```python
from build123d import *

# Parameters (mm, degrees)
FORKED_BLOCK_BODY_DEPTH      = 42.5
SLOT_12X24_DEPTH             = 85
RELIEF_GROOVE_SKETCH_W       = 72
RELIEF_GROOVE_SKETCH_H       = 6
BOTTOM_RELIEF_GROOVE_6_DEPTH = 50
BORE_AND_SADDLE_SKETCH_R     = 12
SADDLE_RECESS_48_DEPTH       = 12
BORE_24_REACH                = 177.873
SKETCH6_3_R                  = 12


with BuildPart() as part:
    # Block Profile Sketch → Forked Block Body (new, symmetric)
    with BuildSketch(Plane(origin=(0, 0, 0), x_dir=(0, 0, -1), z_dir=(1, 0, 0))):
        Polygon((50, 0), (-95, 0), (-95, 90), (-59, 90), (-59, 25), (50, 25), align=None)
    extrude(amount=FORKED_BLOCK_BODY_DEPTH, both=True)

    # Slot Sketch → Slot 12x24 (cut)
    with BuildSketch(Plane(origin=(0, 25, 0), x_dir=(1, 0, 0), z_dir=(0, 1, 0))):
        with BuildLine():
            Line((18.5, 0), (18.5, 50))
            Line((18.5, 50), (-5.5, 50))
            Line((-5.5, 50), (-5.5, 0))
            ThreePointArc((-5.5, 0), (6.5, -12), (18.5, 0))
        make_face()
    extrude(amount=-SLOT_12X24_DEPTH, mode=Mode.SUBTRACT)

    # Relief Groove Sketch → Bottom Relief Groove 6 (cut)
    with BuildSketch(Plane(origin=(42.5, 0, 0), x_dir=(0, 0, -1), z_dir=(1, 0, 0))):
        with Locations((-59, 3)):
            Rectangle(RELIEF_GROOVE_SKETCH_W, RELIEF_GROOVE_SKETCH_H)
    extrude(amount=-BOTTOM_RELIEF_GROOVE_6_DEPTH, mode=Mode.SUBTRACT)

    # Bore and Saddle Sketch → Saddle Recess _48 (cut)
    with BuildSketch(Plane.XY.offset(95)):
        with BuildLine():
            Line((-42.5, 66), (-42.5, 30))
            Line((-42.5, 30), (-24, 30))
            ThreePointArc((-24, 30), (0, 18), (24, 30))
            Line((24, 30), (42.5, 30))
            Line((42.5, 30), (42.5, 66))
            Line((42.5, 66), (24, 66))
            ThreePointArc((24, 66), (0, 78), (-24, 66))
            Line((-24, 66), (-42.5, 66))
        make_face()
        with Locations((0, 48)):
            Circle(BORE_AND_SADDLE_SKETCH_R, mode=Mode.SUBTRACT)
    extrude(amount=-SADDLE_RECESS_48_DEPTH, mode=Mode.SUBTRACT)

    # Sketch6_3 → Bore _24 (cut, up to next)
    with BuildSketch(Plane.XY.offset(95), mode=Mode.PRIVATE) as bore_24_sk1:
        with Locations((0, 48)):
            Circle(SKETCH6_3_R)
    bore_24_tool1 = extrude(bore_24_sk1.sketch, amount=-BORE_24_REACH, mode=Mode.PRIVATE) & part.part
    add(bore_24_tool1.solids().sort_by_distance((0, 48, 95))[0], mode=Mode.SUBTRACT)


solid = part.part
```
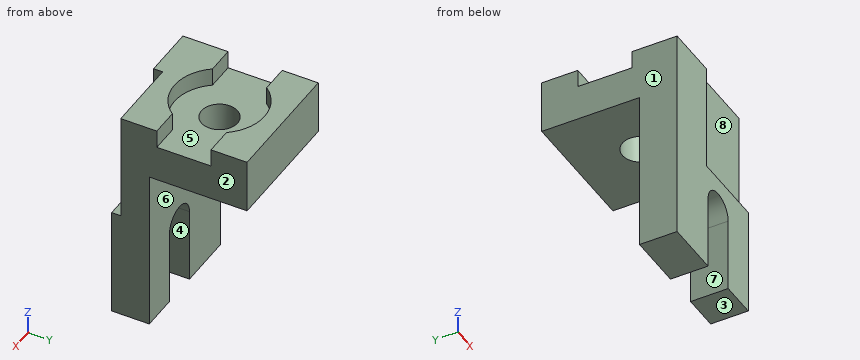
Design review of the part built by this model. Coordinates are the model's own, in mm. Face numbers are marked on the shaded views. A direction names the side the tool comes from. Round coordinates to 2 decimals unless told otherwise and drop trailing zeros. Order: outer loops, then holes, each group sorted by start corner. A loop starts at its lowest first (then second) coordinate and runs counter-clockwise, first axis right, second up. Notation, with made-up numbers: (43.25, -15) - (58.25, -15) arc R7 cw to (58.25, -5) - close; hole circle Ø2 at (-3.5, 55.5). An arc over 180 degrees is marked (long way). Return JSON: item names as keys, results as strings.
Q1. Consider section B-B on z = 26. Write out the cut boundary in (x, y), plus the area to 4 significant figures.
Computed values:
{"outline": "(-42.5, 0) - (-7.5, 0) - (-7.5, 6) - (42.5, 6) - (42.5, 25) - (-42.5, 25) - close", "area": "1,825 mm2"}
Q2. For pin 1 Ø18 at (x, y) = (10.5, 61.5) entering from +Z; pin 2 Ø8 at (x, y) = (12.5, 34) entering from -Z; pin 3 Ø12 at (x, z) = (-26, -25) entering from -Y; pin 4 Ø1.5 at (x, z) = (13.5, 46.5) entering from +Y, all flat-tipped, find the tip position at first contact; note any pin that passes through.
Computed values:
{"pin 1": "stops at z = 83", "pin 2": "stops at z = 59", "pin 3": "stops at y = 0", "pin 4": "stops at y = 25"}
Q3. Machinability: for the marked faces 5, 6, 7 and 8, which of the approach directions +Z, -Z, +X, -X, +Y, -Y give a long, thin tool a straight path to every point of the face, cutting with its end or side? Answer none if there is none.
Computed values:
{"face 5": "+Z", "face 6": "-Z, +X, -X, +Y", "face 7": "-Z, +Y, -Y", "face 8": "+Z, +X, -Y"}
Q4. The part is to be moulded in two halves that separate along X. For the marked faces 1, 2, 3 and 4, say which applies: pulls with the +X half, pulls with the -X half, needs draft (parallel to the pull), parting line crosses it, or undercut.
Computed values:
{"face 1": "pulls with the -X half", "face 2": "pulls with the +X half", "face 3": "needs draft", "face 4": "undercut"}
Q5. Consider section A-A on x = 6.5. Write out the cut boundary in (y, z), plus the area to 3 significant figures.
Computed values:
{"outline": "(0, 12) - (25, 12) - (25, 59) - (37.91, 59) - (37.91, 83) - (18.71, 83) - (18.71, 95) - (6, 95) - (6, 23) - (0, 23) - close; (58.09, 59) - (90, 59) - (90, 95) - (77.29, 95) - (77.29, 83) - (58.09, 83) - close", "area": "2,800 mm2"}
Q6. Wall thickness on L1, parallel to Y at x = 0, z = 68; L2, parallel to Z at x = -14.5, y = 52.5; L3, parallel to Z at x = 25, y = 71.5: over which ranges is each line inside the solid? List them lowest first. Write a range as [from, to].
Computed values:
{"L1": "y = [6, 36], [60, 90]", "L2": "z = [59, 83]", "L3": "z = [59, 95]"}
Q7. Consider section D-D on y = 73. Write out the cut boundary in (x, z), plus the area to 3 significant figures.
Computed values:
{"outline": "(-42.5, 59) - (42.5, 59) - (42.5, 95) - (16.58, 95) - (16.58, 83) - (-16.58, 83) - (-16.58, 95) - (-42.5, 95) - close", "area": "2,660 mm2"}
Q8. Consider section C-C on x = 34. Write out the cut boundary in (y, z), plus the area to 3 significant figures.
Computed values:
{"outline": "(0, -50) - (25, -50) - (25, 59) - (90, 59) - (90, 95) - (66, 95) - (66, 83) - (30, 83) - (30, 95) - (6, 95) - (6, 23) - (0, 23) - close", "area": "5,100 mm2"}
